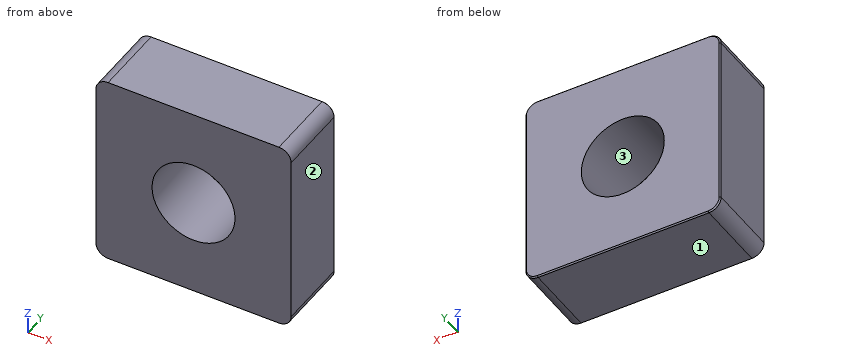
from build123d import *

# Parameters (mm, degrees)
SKETCH1_W              = 80
SKETCH1_H              = 80
BOSS_EXTRUDE1_DEPTH    = 30
M36X2_0_TAPPED_HOLE1_D = 34
FILLET1_R              = 5
CHAMFER1_SIZE          = 0.5


with BuildPart() as part:
    # Sketch1 → Boss-Extrude1 (new body)
    with BuildSketch(Plane(origin=(0, 30, 0), x_dir=(1, 0, 0), z_dir=(0, 1, 0))):
        Rectangle(SKETCH1_W, SKETCH1_H)
    extrude(amount=-BOSS_EXTRUDE1_DEPTH)

    # M36x2.0 Tapped Hole1 (through all)
    with Locations(Plane(origin=(0, 30, 0), x_dir=(1, 0, 0), z_dir=(0, 1, 0))):
        with Locations((0, 0)):
            Hole(M36X2_0_TAPPED_HOLE1_D / 2)

    # Fillet1
    fillet1_edges = [part.edges().sort_by_distance(p)[0] for p in [
        (-40, 15, -40),
        (40, 15, -40),
        (40, 15, 40),
        (-40, 15, 40),
    ]]
    fillet(fillet1_edges, radius=FILLET1_R)

    # Chamfer1
    chamfer1_edges = [part.edges().sort_by_distance(p)[0] for p in [
        (0, 30, 40),
        (-40, 30, 0),
        (40, 30, 0),
        (0, 30, -40),
        (-38.535533906, 30, -38.535533906),
        (38.535533906, 30, -38.535533906),
        (-38.535533906, 30, 38.535533906),
        (38.535533906, 30, 38.535533906),
    ]]
    chamfer(chamfer1_edges, length=CHAMFER1_SIZE)


solid = part.part
The listing builds one solid part. Answer for the finished solid, in the listing's coordinates (mm). Face numbers are marked on the shaded views. Give positions to 0.01 mm unless a question says otherwise; leave off trailing zeros. Write each loop counter-clockwise with the first axis right and the second up, starting at its lowest first coordinate (ties: lowest second). Pieces come first, ordered by that corner, then holes. Notation, with made-up numbers: (-11, 45.5) - (19, 45.5) arc R24 ccw to (19, 67.5) - close; hole circle Ø5 at (-25, 54). An arc over 180 degrees is marked (long way). Use a Markdown table: item, result.
1. Section C-C on z = 0 is taken. Write down the section's boundary in (x, y), plus the area to 3 significant figures.
Values follow:
| item | result |
|---|---|
| outline | (-40, 0) - (-17, 0) - (-17, 30) - (-39.5, 30) - (-40, 29.5) - close; (17, 0) - (40, 0) - (40, 29.5) - (39.5, 30) - (17, 30) - close |
| area | 1,380 mm² |
2. Section A-A on x = 8 is taken. Write down the section's boundary in (y, z), plus the area to 3 significant figures.
Values follow:
| item | result |
|---|---|
| outline | (0, -40) - (29.5, -40) - (30, -39.5) - (30, -15) - (0, -15) - close; (0, 15) - (30, 15) - (30, 39.5) - (29.5, 40) - (0, 40) - close |
| area | 1,500 mm² |
3. Section B-B on y = 3 is taken. Write down the section's boundary in (x, z).
Values follow:
| item | result |
|---|---|
| outline | (-40, -35) arc R5 ccw to (-35, -40) - (35, -40) arc R5 ccw to (40, -35) - (40, 35) arc R5 ccw to (35, 40) - (-35, 40) arc R5 ccw to (-40, 35) - close; hole circle Ø34 at (0, 0) |
4. This flat-tipped pin is pushed along its axis until it touches: P1, Ø1, axis at x = -14, z = 8, coming from the +Y side. Where does it stop, or does it pass through?
Values follow:
| item | result |
|---|---|
| P1 | passes through |
5. Find the intervals of material crossed by probe 1 along X at (y, z) = (26.5, -0.5); probe 2 along Z at (x, y) = (0, 20); probe 3 along Z at (x, y) = (7.5, 27.75), in increasing order. Write a range as from..to.
Values follow:
| item | result |
|---|---|
| probe 1 | x = -40..-16.99, 16.99..40 |
| probe 2 | z = -40..-17, 17..40 |
| probe 3 | z = -40..-15.26, 15.26..40 |
6. For a pull along Z with two mould halves and no side action, classify the marked faces 1, 2 and 3 as released by +Z, released by -Z, zero draft, split by the parting line, or undercut.
Values follow:
| item | result |
|---|---|
| face 1 | released by -Z |
| face 2 | zero draft |
| face 3 | undercut |
